Design review of the part shown in the three views and the two pictorial views. Dimensions are in mm from the part's minimum x, y and z. Coordinates: 2 decimals unless noted, no trailing zeros. Write each loop counter-clockwise with the first axis right and the second up, starting at its lowest first coordinate (ties: lowest second). Pieces come first, ordered by that corner, then holes. Notation, with made-up numbers: M -22,58.5 L 20,58.5 A11 ccw 20,67.5 Z; hole C 50,-19.75 d1. An arc over 180 degrees is marked long. One line per question, with ' | ' between items.
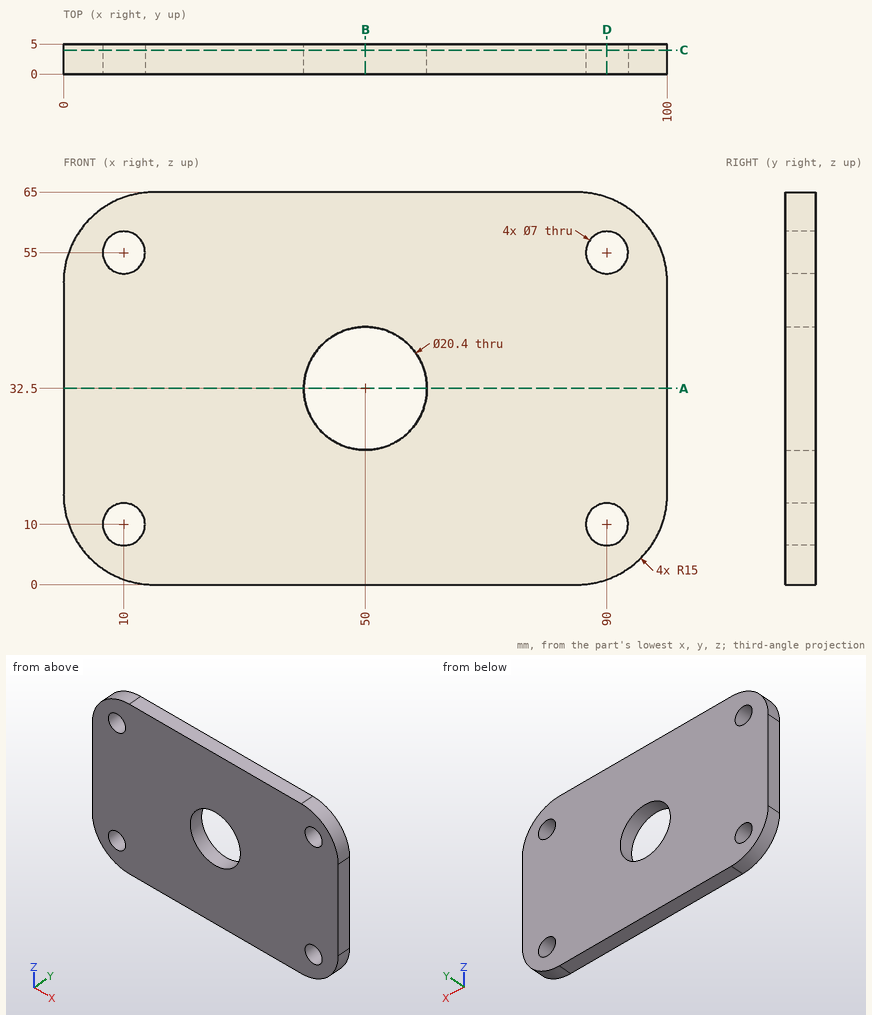
1. For line 1 along Z through (x, y) = (9.5, 1.5); line 2 along X through (y, z) = (1.6, 32); line 3 along X through (y, z) = (2.1, 55), list the stretches that pass through material, from the lowest coordinate up.
Computed values:
line 1: z = 1.04 to 6.54, 13.46 to 51.54, 58.46 to 63.96 | line 2: x = 0 to 39.81, 60.19 to 100 | line 3: x = 0.86 to 6.5, 13.5 to 86.5, 93.5 to 99.14
2. Take a section at D-D on x = 90. State the section outline as (y, z) points, plus the area to 3 significant figures.
Computed values:
outline: M 0,0.86 L 5,0.86 L 5,6.5 L 0,6.5 Z; M 0,13.5 L 5,13.5 L 5,51.5 L 0,51.5 Z; M 0,58.5 L 5,58.5 L 5,64.14 L 0,64.14 Z | area: 246 mm2
3. Take a section at C-C on y = 4. State the section outline as (x, z) points, plus the area to 3 significant figures.
Computed values:
outline: M 0,15 A15 ccw 15,0 L 85,0 A15 ccw 100,15 L 100,50 A15 ccw 85,65 L 15,65 A15 ccw 0,50 Z; hole C 10,10 d7; hole C 10,55 d7; hole C 50,32.5 d20.4; hole C 90,10 d7; hole C 90,55 d7 | area: 5,830 mm2
4. Clearance check with a flat-ended pin moving along its axis: P1, Ø4, axis at x = 10, z = 55, coming from the -Y side. State where the tip first meets the part, or that it passes through.
Computed values:
P1: passes through
5. Take a section at B-B on x = 50. State the section outline as (y, z) points.
Computed values:
outline: M 0,0 L 5,0 L 5,22.3 L 0,22.3 Z; M 0,42.7 L 5,42.7 L 5,65 L 0,65 Z
6. Take a section at A-A on z = 32.5. State the section outline as (x, y) points, plus the area to 3 significant figures.
Computed values:
outline: M 0,0 L 39.8,0 L 39.8,5 L 0,5 Z; M 60.2,0 L 100,0 L 100,5 L 60.2,5 Z | area: 398 mm2
